from build123d import *

# Parameters (mm, degrees)
BOSS_EXTRUDE1_DEPTH = 20
SKETCH3_OUTSIDE_W   = 31.822
SKETCH3_OUTSIDE_H   = 35.226
SKETCH3_OUTSIDE_R   = 10.5
CUT_EXTRUDE1_DEPTH  = 15
CHAMFER1_SIZE       = 1
M10_TAPPED_HOLE1_D  = 8.5


with BuildPart() as part:
    # Sketch1 → Boss-Extrude1 (new body)
    with BuildSketch(Plane(origin=(0, 0, 0), x_dir=(1, 0, 0), z_dir=(0, 1, 0))):
        Polygon((11, -6.350852961), (11, 6.350852961), (0, 12.701705922), (-11, 6.350852961), (-11, -6.350852961), (0, -12.701705922), align=None)
    extrude(amount=BOSS_EXTRUDE1_DEPTH)

    # Sketch3 outside → Cut-Extrude1 (cut)
    with BuildSketch(Plane.XZ):
        Rectangle(SKETCH3_OUTSIDE_W, SKETCH3_OUTSIDE_H)
        with Locations(Location((0, 0, 0), (0, 0, 270))):
            Circle(SKETCH3_OUTSIDE_R, mode=Mode.SUBTRACT)
    extrude(amount=-CUT_EXTRUDE1_DEPTH, mode=Mode.SUBTRACT)

    # Chamfer1
    chamfer1_edges = [part.edges().sort_by_distance(p)[0] for p in [
        (0, 0, 10.5),
    ]]
    chamfer(chamfer1_edges, length=CHAMFER1_SIZE)

    # M10 Tapped Hole1 (through all)
    with Locations(Plane.ZX.offset(20)):
        with Locations((0, 0)):
            Hole(M10_TAPPED_HOLE1_D / 2)


solid = part.part
Check sheet for the modelled part. Datum: model origin and axes. Units: mm. A direction names the side the tool comes from. Round coordinates to 2 decimals unless told otherwise and drop trailing zeros. Order: outer loops, then holes, each group sorted by start corner. A loop starts at its lowest first (then second) coordinate and runs counter-clockwise, first axis right, second up.
(1) Cross-section at C-C, the plane y = 6. Enter the section's corners in (x, z), and give its area (3 significant figures).
(2) Draft check along X on faces 1 (the cylindrical face through (3.584, 9.86, -2.285)), 2 (the flat face through (11, 17, 0)), 3 (the flat face through (4, 0, 2)), 4 (the flat face through (-11, 17, 0)). Enter one of: pulls with the +X half, pulls with the -X half, needs draft (parallel to the pull), parting line crosses it, or undercut.
(3) Cross-section at A-A, the plane z = 0. Enter the section's corners in (x, y).
(4) Go/stop test with flat-tipped pins: P1, Ø2, axis at x = 5.5, y = 11, coming from the +Z side; P2, Ø8, axis at x = 4, y = 14.5, coming from the -Z side. Record where each tip stops, or that it passes through.
(5) Scan lines: probe 1 along X at (y, z) = (11, 0); probe 2 along Y at (x, z) = (-2.25, 10.75); probe 3 along Z at (x, y) = (0.25, 17.25). Record each from-to range of solid material in increasing order.
(6) Cross-section at B-B, the plane y = 16.5. Enter the section's corners in (x, z), and give its area (3 significant figures).
(7) Access from +Z, -Z, +X, -X, +Y, -Y to the whole of each face (thin tool, end or side, straight path). Record for faces 5 (the cylindrical face through (3.2, 7.9, -10)), 6 (the flat face through (0, 20, 5)).
Check sheet entries:
1. outline: circle Ø21 at (0, 0); hole circle Ø8.5 at (0, 0)
1. area: 290 mm2
2. face 1: undercut
2. face 2: pulls with the +X half
2. face 3: needs draft
2. face 4: pulls with the -X half
3. outline: (-11, 15) - (-10.5, 15) - (-10.5, 1) - (-9.5, 0) - (-4.25, 0) - (-4.25, 20) - (-11, 20) - close; (4.25, 0) - (9.5, 0) - (10.5, 1) - (10.5, 15) - (11, 15) - (11, 20) - (4.25, 20) - close
4. P1: stops at z = 9.49
4. P2: stops at z = -12.68
5. probe 1: x = -10.5 to -4.25, 4.25 to 10.5
5. probe 2: y = 15 to 20
5. probe 3: z = -12.56 to -4.24, 4.24 to 12.56
6. outline: (-11, -6.35) - (0, -12.7) - (11, -6.35) - (11, 6.35) - (0, 12.7) - (-11, 6.35) - close; hole circle Ø8.5 at (0, 0)
6. area: 362 mm2
7. face 5: -Y
7. face 6: +Z, -Z, +X, -X, +Y
